Check sheet for the drawn part. Datum: minimum x, y, z corner. Units: mm. A direction names the side the tool comes from. Give positions to 0.01 mm unless a question says otherwise; leave off trailing zeros. Loops run counter-clockwise (first coordinate to the right, second up) from the corner with the lowest first, then second, coordinate; pieces in that order, holes last. Notation, with made-up numbers: (82.5, 33.25) - (89.5, 33.25) arc R22 cw to (89.5, 45.25) - close; hole circle Ø3 at (89, 56.25). An arc over 180 degrees is marked (long way). One line per item, written item: value. Start each with the question number.
1. Sectioned sample at C-C (z = 10). Record the cut outline in (x, y), plus the area to 3 significant figures.
2. Scan lines: L1, parallel to X at y = 37.25, z = 10; L2, parallel to Z at x = 103, y = 35; L3, parallel to Z at x = 55, y = 5. Record each from-to range of solid material in increasing order. Write a range as [from, to].
3. Sectioned sample at B-B (x = 19.5). Record the cut outline in (y, z).
4. Mould release check, pull along Z, two halves, no side actions. Record for the marked faces 3, 4 and 5: pulls with the +Z half, pulls with the -Z half, needs draft (parallel to the pull), parting line crosses it, or undercut.
5. Sectioned sample at A-A (y = 12.5). Record the cut outline in (x, z).
6. Gauge pin test, flat ends, axial feed: pin 1 (6 mm diameter, centred on x = 35.5, z = 20, fed in from -Y); pin 2 (2.5 mm diameter, centred on x = 30.5, z = 10, fed in from +Y). Record the tip position at first contact, or that the pin passes through.
7. Sectioned sample at D-D (x = 33). Record the cut outline in (y, z).
8. Access from +Z, -Z, +X, -X, +Y, -Y to the whole of each face (thin tool, end or side, straight path). Record for the marked faces 1 and 2.
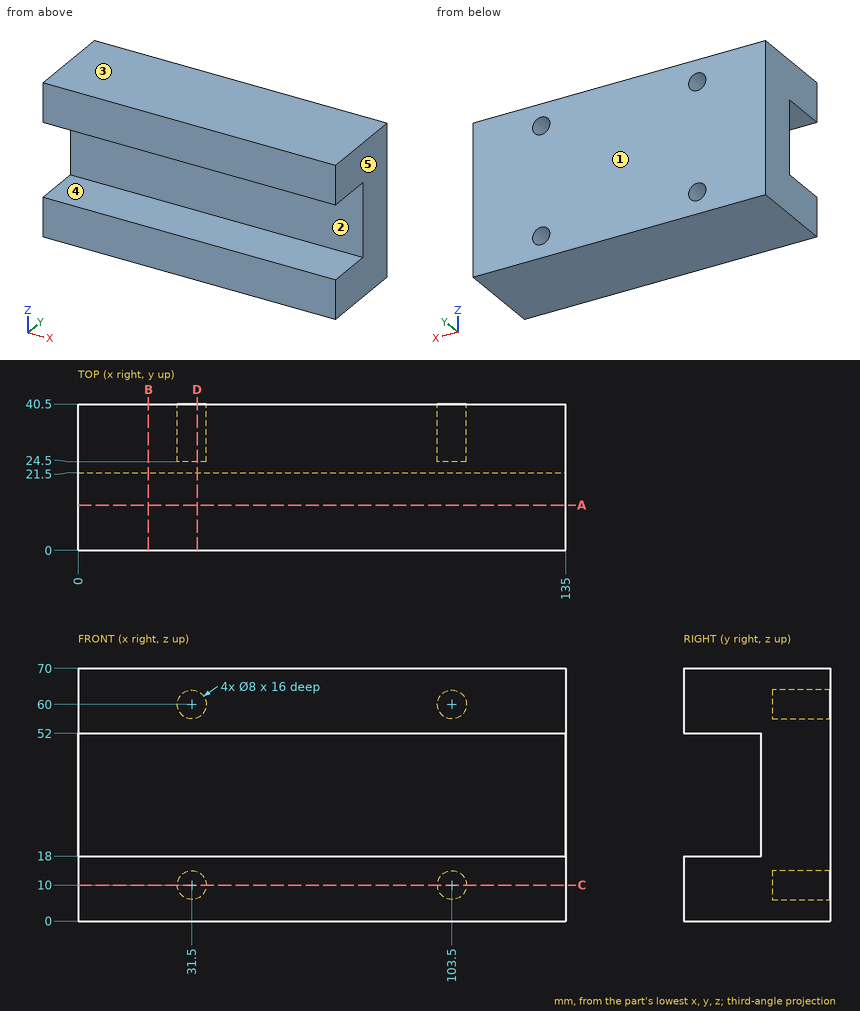
Results are:
1. outline: (0, 0) - (135, 0) - (135, 40.5) - (107.5, 40.5) - (107.5, 24.5) - (99.5, 24.5) - (99.5, 40.5) - (35.5, 40.5) - (35.5, 24.5) - (27.5, 24.5) - (27.5, 40.5) - (0, 40.5) - close
1. area: 5,210 mm^2
2. L1: x = [0, 27.5], [35.5, 99.5], [107.5, 135]
2. L2: z = [0, 6.03], [13.97, 56.03], [63.97, 70]
2. L3: z = [0, 18], [52, 70]
3. outline: (0, 0) - (40.5, 0) - (40.5, 70) - (0, 70) - (0, 52) - (21.5, 52) - (21.5, 18) - (0, 18) - close
4. face 3: pulls with the +Z half
4. face 4: undercut
4. face 5: needs draft
5. outline: (0, 0) - (135, 0) - (135, 18) - (0, 18) - close; (0, 52) - (135, 52) - (135, 70) - (0, 70) - close
6. pin 1: stops at y = 0
6. pin 2: stops at y = 24.5
7. outline: (0, 0) - (40.5, 0) - (40.5, 6.29) - (24.5, 6.29) - (24.5, 13.71) - (40.5, 13.71) - (40.5, 56.29) - (24.5, 56.29) - (24.5, 63.71) - (40.5, 63.71) - (40.5, 70) - (0, 70) - (0, 52) - (21.5, 52) - (21.5, 18) - (0, 18) - close
8. face 1: +Z, -Z, +X, -X, +Y
8. face 2: +X, -X, -Y
